```python
from build123d import *

# Parameters (mm, degrees)
BRACKET_BODY_DEPTH      = 40
FRONT_BORE_SKETCH_R     = 9.403768256
FRONT_BORE_DEPTH        = 105.043260233
FLANGE_NOTCH_SKETCH_W   = 8
FLANGE_NOTCH_SKETCH_H   = 18
FLANGE_NOTCH_CUTS_DEPTH = 40
FLANGE_SLOT_SKETCH_W    = 8
FLANGE_SLOT_SKETCH_H    = 18
FLANGE_SLOT_CUT_DEPTH   = 40
CROSS_HOLE_SKETCH_R     = 7
CROSS_HOLE_14_DEPTH     = 105.043260233


with BuildPart() as part:
    # Bracket Profile Sketch → Bracket Body (new body)
    with BuildSketch(Plane.XY):
        Polygon((0, 0), (50, 0), (50, 15), (75, 15), (75, 25), (50, 25), (50, 47), (40, 60), (15, 60), (0, 47), (0, 25), (-25, 25), (-25, 15), (0, 15), align=None)
    extrude(amount=BRACKET_BODY_DEPTH)

    # Front Bore Sketch → Front Bore (cut, through all)
    with BuildSketch(Plane.XY.offset(40)):
        with Locations((27.5, 30)):
            Circle(FRONT_BORE_SKETCH_R)
    extrude(amount=-FRONT_BORE_DEPTH, mode=Mode.SUBTRACT)

    # Flange Notch Sketch → Flange Notch Cuts (cut)
    with BuildSketch(Plane(origin=(0, 25, 0), x_dir=(1, 0, 0), z_dir=(0, 1, 0))):
        with Locations((71, -20)):
            Rectangle(FLANGE_NOTCH_SKETCH_W, FLANGE_NOTCH_SKETCH_H)
    extrude(amount=-FLANGE_NOTCH_CUTS_DEPTH, mode=Mode.SUBTRACT)

    # Flange Slot Sketch → Flange Slot Cut (cut)
    with BuildSketch(Plane(origin=(0, 25, 0), x_dir=(1, 0, 0), z_dir=(0, 1, 0))):
        with Locations((-21, -20)):
            Rectangle(FLANGE_SLOT_SKETCH_W, FLANGE_SLOT_SKETCH_H)
    extrude(amount=-FLANGE_SLOT_CUT_DEPTH, mode=Mode.SUBTRACT)

    # Cross Hole Sketch → Cross Hole Ø14 (cut, through all)
    with BuildSketch(Plane(origin=(50, 0, 0), x_dir=(0, 0, -1), z_dir=(1, 0, 0))):
        with Locations((-20, 36)):
            Circle(CROSS_HOLE_SKETCH_R)
    extrude(amount=-CROSS_HOLE_14_DEPTH, mode=Mode.SUBTRACT)


solid = part.part
```
Can you work these out from the model? Positions are in its coordinate system, mm. A direction names the side the tool comes from. Coordinates: 2 decimals unless noted, no trailing zeros. Loops run counter-clockwise (first coordinate to the right, second up) from the corner with the lowest first, then second, coordinate; pieces in that order, holes last. Notation, with made-up numbers: M 15.25,22.5 L 61.25,22.5 A35 cw 61.25,56.5 Z; hole C -35.75,66 d10. An arc over 180 degrees is marked long. Put each result on its own line as item: value. Start each with the question number.
(1) I need wall thicknesses on probe 1 along Y at (x, z) = (17, 20); probe 2 along Y at (x, z) = (27, 28); probe 3 along Z at (x, y) = (16, 36). Which ranges of each line are inside material? Lowest first, please.
(2) Imagine slicing it at D-D on z = 20. List the corners of the cut face in (x, y) for me.
(3) Which directions (+Z, -Z, +X, -X, +Y, -Y) give clear straight access to the entire face, cutting with the end or side of a thin tool? Please do faces 5 (the face through (60, 25, 20)), 6 (the face through (71, 20, 11)), 7 (the face through (60, 15, 20)).
(4) Imagine slicing it at C-C on y = 35. List the corners of the cut face in (x, z) for me.
(5) We'd pull the mould along Z, two halves only. Please class faces 1 (the face through (24, 17, 0)), 2 (the face through (-21, 20, 29)), 3 (the face through (7.605, 53.591, 19.72)), 4 (the face through (71, 20, 29)): +Z half, -Z half, draft (parallel to the pull), parting line (faces both ways), or undercut.
(6) Will these pins go through, and if not, where does the flat tip stop? pin 1 Ø17.5 at (y, z) = (40.5, 29.5) entering from -X; pin 2 Ø8 at (y, z) = (18, 20) entering from -X; pin 3 Ø11 at (y, z) = (18, 19.5) entering from +X.
(7) Imagine slicing it at A-A on z = 5. List the corners of the cut face in (x, y) for me.
(8) Imagine slicing it at B-B on x = -18. List the corners of the cut face in (y, z) for me.
Worked answers:
1. probe 1: y = 0 to 29, 43 to 60
1. probe 2: y = 0 to 20.61, 39.39 to 60
1. probe 3: z = 0 to 13, 27 to 40
2. outline: M -17,15 L 0,15 L 0,0 L 50,0 L 50,15 L 67,15 L 67,25 L 50,25 L 50,29 L 36.85,29 A9.4 cw 18.15,29 L 0,29 L 0,25 L -17,25 Z; M 0,43 L 50,43 L 50,47 L 40,60 L 15,60 L 0,47 Z
3. face 5: +Z, -Z, +X, +Y
3. face 6: +X, +Y, -Y
3. face 7: +Z, -Z, +X, -Y
4. outline: M 0,0 L 19.54,0 L 19.54,13.07 L 0,13.07 Z; M 0,26.93 L 19.54,26.93 L 19.54,40 L 0,40 Z; M 35.46,0 L 50,0 L 50,13.07 L 35.46,13.07 Z; M 35.46,26.93 L 50,26.93 L 50,40 L 35.46,40 Z
5. face 1: -Z half
5. face 2: undercut
5. face 3: draft
5. face 4: undercut
6. pin 1: stops at x = 0
6. pin 2: stops at x = -17
6. pin 3: stops at x = 67
7. outline: M -25,15 L 0,15 L 0,0 L 50,0 L 50,15 L 75,15 L 75,25 L 50,25 L 50,47 L 40,60 L 15,60 L 0,47 L 0,25 L -25,25 Z; hole C 27.5,30 d18.81
8. outline: M 15,0 L 25,0 L 25,11 L 15,11 Z; M 15,29 L 25,29 L 25,40 L 15,40 Z
